Can you work these out from the model? Positions are in its coordinate system, mm. A direction names the side the tool comes from. Give positions to 0.01 mm unless a question says otherwise; leave off trailing zeros. Loops run counter-clockwise (first coordinate to the right, second up) from the corner with the lowest first, then second, coordinate; pieces in that order, holes last. Notation, with made-up numbers: M -5.5,-10.5 L 42.5,-10.5 A30 cw 42.5,21.5 Z; hole C 48.25,66 d10. An arc over 180 degrees is marked long. Answer as a JSON object with one key per item and string values.
```python
from build123d import *

# Parameters (mm, degrees)
SKETCH_1_R          = 2
SKETCH_1_R_2        = 1.55
SKETCH_1_R_3        = 10
SKETCH_1_R_4        = 6
EXTRUDE_1_DEPTH     = 6
CUT_EXTRUDE_1_DEPTH = 59.180752831
FILLET_1_R          = 1


with BuildPart() as part:
    # 草图1 → 凸台-拉伸1 (new body)
    with BuildSketch(Plane.XY):
        with BuildLine():
            Line((46.777777778, 9.840706589), (3.2, 17.71327186))
            ThreePointArc((3.2, 17.71327186), (-18, 0), (3.2, -17.71327186))
            Line((3.2, -17.71327186), (46.777777778, -9.840706589))
            ThreePointArc((46.777777778, -9.840706589), (55, 0), (46.777777778, 9.840706589))
        make_face()
        with Locations((0, 13.5)):
            Circle(SKETCH_1_R, mode=Mode.SUBTRACT)
        with Locations((6.75, 11.691342951)):
            Circle(SKETCH_1_R_2, mode=Mode.SUBTRACT)
        with Locations((0, -13.5)):
            Circle(SKETCH_1_R, mode=Mode.SUBTRACT)
        with Locations((-6.75, -11.691342951)):
            Circle(SKETCH_1_R_2, mode=Mode.SUBTRACT)
        with Locations((6.75, -11.691342951)):
            Circle(SKETCH_1_R_2, mode=Mode.SUBTRACT)
        with Locations((-11.691342951, -6.75)):
            Circle(SKETCH_1_R, mode=Mode.SUBTRACT)
        with Locations((11.691342951, -6.75)):
            Circle(SKETCH_1_R, mode=Mode.SUBTRACT)
        with Locations((-13.5, 0)):
            Circle(SKETCH_1_R_2, mode=Mode.SUBTRACT)
        Circle(SKETCH_1_R_3, mode=Mode.SUBTRACT)
        with Locations((-11.691342951, 6.75)):
            Circle(SKETCH_1_R, mode=Mode.SUBTRACT)
        with Locations((13.5, 0)):
            Circle(SKETCH_1_R_2, mode=Mode.SUBTRACT)
        with Locations((11.691342951, 6.75)):
            Circle(SKETCH_1_R, mode=Mode.SUBTRACT)
        with Locations((-6.75, 11.691342951)):
            Circle(SKETCH_1_R_2, mode=Mode.SUBTRACT)
        with Locations((45, 0)):
            Circle(SKETCH_1_R_4, mode=Mode.SUBTRACT)
    extrude(amount=EXTRUDE_1_DEPTH)

    # 草图3 → 切除-拉伸1 (cut, through all)
    with BuildSketch(Plane.XY.offset(6)):
        with BuildLine():
            Line((37.366586992, 6.459954012), (14.562692012, 10.579603082))
            ThreePointArc((14.562692012, 10.579603082), (17.119118789, 5.561993518), (18, 0))
            Line((18, 0), (35, 0))
            ThreePointArc((35, 0), (35.610268106, 3.439903336), (37.366586992, 6.459954012))
        make_face()
        with BuildLine():
            Line((35, 0), (18, 0))
            ThreePointArc((18, 0), (17.119118789, -5.561993518), (14.562692012, -10.579603082))
            Line((14.562692012, -10.579603082), (37.366586992, -6.459954012))
            ThreePointArc((37.366586992, -6.459954012), (35.610268106, -3.439903336), (35, 0))
        make_face()
    extrude(amount=-CUT_EXTRUDE_1_DEPTH, mode=Mode.SUBTRACT)

    # 圆角1
    fillet_1_edges = [part.edges().sort_by_distance(p)[0] for p in [
        (14.562692012, -10.579603082, 3),
        (14.562692012, 10.579603082, 3),
        (37.366586992, 6.459954012, 3),
        (37.366586992, -6.459954012, 3),
    ]]
    fillet(fillet_1_edges, radius=FILLET_1_R)


solid = part.part
```
1) Suppose I cut it at A-A, the plane x = 0. Write out the boundary of the cut face in (y, z), and give its area (3 significant figures).
Answer list:
{"outline": "M -18,0 L -15.5,0 L -15.5,6 L -18,6 Z; M -11.5,0 L -10,0 L -10,6 L -11.5,6 Z; M 10,0 L 11.5,0 L 11.5,6 L 10,6 Z; M 15.5,0 L 18,0 L 18,6 L 15.5,6 Z", "area": "48.0 mm^2"}
2) If we mould it in two halves opening along X, with no side actions, what happens to faces 3 (the cylindrical face through (9.693, 6.838, 2.958)), 4 (the flat face through (10, -4, 6)), 5 (the flat face through (24.684, -13.832, 2.958))? For each: +X half, -X half, draft (parallel to the pull), parting line (faces both ways), or undercut.
Answer list:
{"face 3": "undercut", "face 4": "draft", "face 5": "+X half"}
3) Please list where these lines run through material, in increasing order: line 1 along Y through (x, z) = (0, 4.5); line 2 along X through (y, z) = (-6.5, 0.45); line 3 along Y through (x, z) = (-1.5, 5.2). Write a range as from..to.
Answer list:
{"line 1": "-18..-15.5, -11.5..-10, 10..11.5, 15.5..18", "line 2": "-16.79..-13.68, -9.71..-7.6, 7.6..9.71, 13.68..16.79, 36.3..52.6", "line 3": "-17.94..-14.82, -12.18..-9.89, 9.89..12.18, 14.82..17.94"}
4) Will these pins go through, and if not, where does the flat tip stop? pin 1 Ø3 at (x, z) = (31, 4.5) entering from +Y; pin 2 Ø2 at (y, z) = (-3.5, 3) entering from -X; pin 3 Ø1 at (x, z) = (-1.5, 3.5) entering from +Y.
Answer list:
{"pin 1": "y = 12.96", "pin 2": "x = -17.83", "pin 3": "y = 17.97"}
5) Suppose I cut it at C-C, the plane z = 2.1. Give the number of separate pieces and of enclosed holes in the cut face, and give its area (3 significant figures).
Answer list:
{"separate pieces": "1", "enclosed holes": "15", "area": "1,080 mm^2"}
6) For faces 1 (the cylindrical face through (55, 0, 3)), 2 (the flat face through (26.173, -8.482, 3.042)), which set-ups out of +Z, -Z, +X, -X, +Y, -Y let a thin tool reach every point of the face, with its end or its side?
Answer list:
{"face 1": "+Z, -Z, +X", "face 2": "+Z, -Z"}
7) Suppose I cut it at D-D, the plane y = 8. Write out the boundary of the cut face in (x, z), and give its area (3 significant figures).
Answer list:
{"outline": "M -16.12,0 L -13.25,0 L -13.25,6 L -16.12,6 Z; M -10.13,0 L -6,0 L -6,6 L -10.13,6 Z; M 6,0 L 10.13,0 L 10.13,6 L 6,6 Z; M 13.25,0 L 16.12,0 L 16.12,6 L 13.25,6 Z; M 28.84,0 L 51,0 L 51,6 L 28.84,6 Z", "area": "217 mm^2"}
8) Suppose I cut it at B-B, the plane x = 45. Write out the boundary of the cut face in (y, z).
Answer list:
{"outline": "M -10.16,0 L -6,0 L -6,6 L -10.16,6 Z; M 6,0 L 10.16,0 L 10.16,6 L 6,6 Z"}
